For this review, use the dimensioned drawing (mm, ordinates from the lowest corner) and the shaded views. Coordinates: 2 decimals unless noted, no trailing zeros. Write each loop counter-clockwise with the first axis right and the second up, starting at its lowest first coordinate (ties: lowest second). Pieces come first, ordered by that corner, then holes. Notation, with made-up numbers: M -30.5,21.5 L 3.5,21.5 A23 cw 3.5,36.5 Z; hole C -10.75,30.25 d9. An arc over 180 degrees is marked long. One line per question, with ' | ' between items.
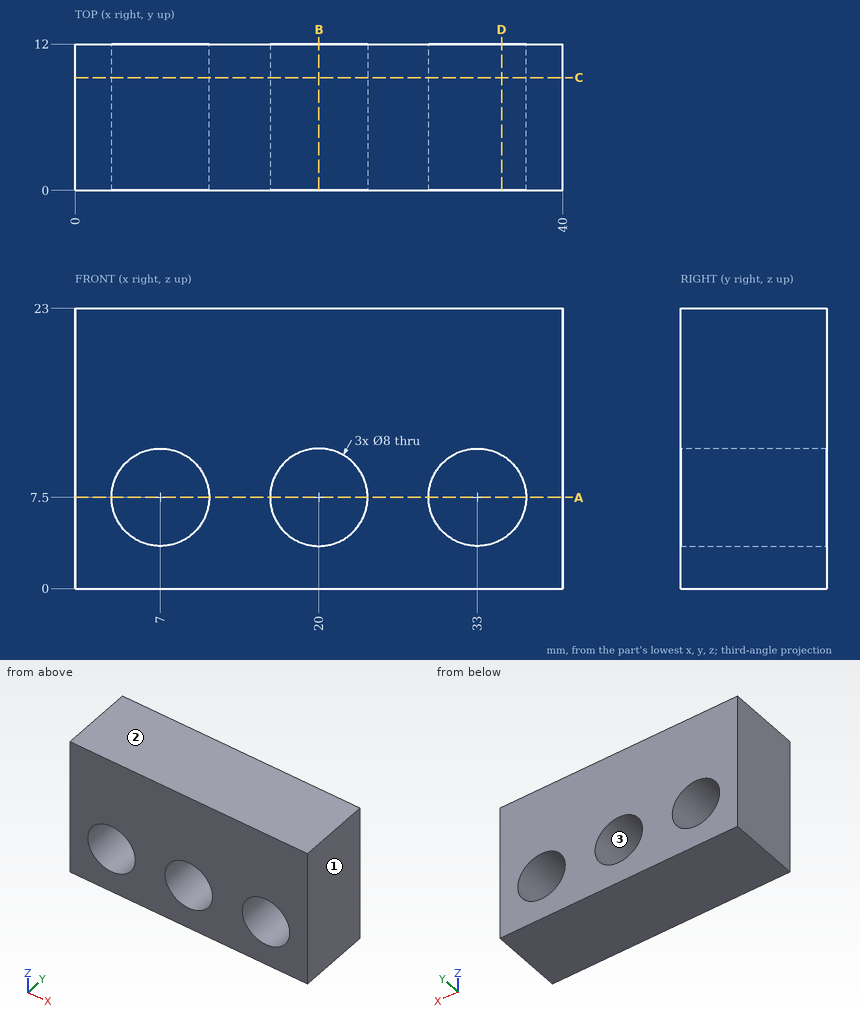
1) We need section B-B on x = 20. State the section outline as (y, z) points.
Responses:
outline: M 0,0 L 12,0 L 12,3.5 L 0,3.5 Z; M 0,11.5 L 12,11.5 L 12,23 L 0,23 Z
2) We need section D-D on x = 35. State the section outline as (y, z) points, then the cut area to 3 significant figures.
Responses:
outline: M 0,0 L 12,0 L 12,4.04 L 0,4.04 Z; M 0,10.96 L 12,10.96 L 12,23 L 0,23 Z | area: 193 mm^2
3) The part is to be moulded in two halves that separate along Z. For the marked faces 1, 2 and 3, say which applies: +Z half, -Z half, draft (parallel to the pull), parting line (faces both ways), or undercut.
Responses:
face 1: draft | face 2: +Z half | face 3: undercut
4) To check wall thickness, follow line 1 along X through (y, z) = (7.5, 7.5); line 2 along X through (y, z) = (1, 5.25); line 3 along Z through (x, y) = (22, 2). State the ranges of each line that lie inside material, in increasing order. Write a range as [from, to].
Responses:
line 1: [0, 3], [11, 16], [24, 29], [37, 40] | line 2: [0, 3.69], [10.31, 16.69], [23.31, 29.69], [36.31, 40] | line 3: [0, 4.04], [10.96, 23]
5) Insertion check: pin 1 Ø4 at (x, z) = (34.5, 14) entering from -Y; pin 2 Ø5 at (x, z) = (33, 7.5) entering from +Y. Each pin has a flat end and moves straight along its axis. Give the tip position at first contact, or say it passes through.
Responses:
pin 1: y = 0 | pin 2: through
6) We need section C-C on y = 9.25. State the section outline as (x, z) points.
Responses:
outline: M 0,0 L 40,0 L 40,23 L 0,23 Z; hole C 7,7.5 d8; hole C 20,7.5 d8; hole C 33,7.5 d8
7) We need section A-A on z = 7.5. State the section outline as (x, y) points.
Responses:
outline: M 0,0 L 3,0 L 3,12 L 0,12 Z; M 11,0 L 16,0 L 16,12 L 11,12 Z; M 24,0 L 29,0 L 29,12 L 24,12 Z; M 37,0 L 40,0 L 40,12 L 37,12 Z
